Can you work these out from the model? Positions are in its coordinate system, mm. Give positions to 0.01 mm unless a question says otherwise; leave off trailing zeros. Loops run counter-clockwise (first coordinate to the right, second up) from the corner with the lowest first, then second, coordinate; pieces in that order, holes last. Notation, with made-up numbers: M -32.5,34.25 L -13.5,34.25 A22 cw -13.5,68.25 Z; hole C -8.5,10 d1. An arc over 180 degrees is marked long. Answer as a JSON object with one key per item and string values.
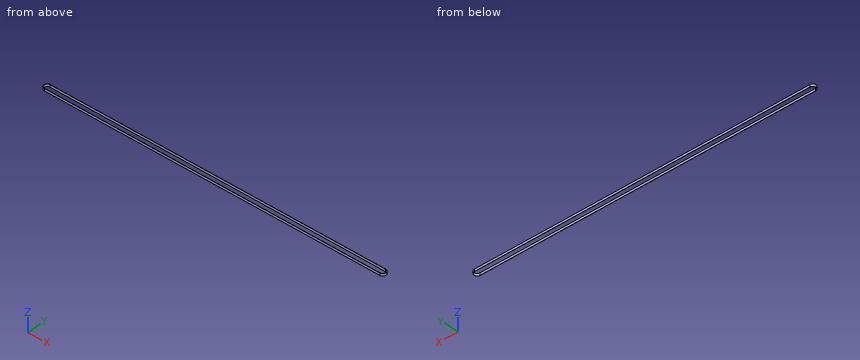
```python
from build123d import *

# Parameters (mm, degrees)
EXTRUDE_1_DEPTH = 7.5


with BuildPart() as part:
    # 草图2 → 拉伸-薄壁1 (new, symmetric)
    with BuildSketch(Plane.XY):
        with BuildLine():
            Line((2155, -20.415), (0, -20.415))
            ThreePointArc((0, -20.415), (-20.415, 0), (0, 20.415))
            Line((0, 20.415), (2155, 20.415))
            ThreePointArc((2155, 20.415), (2175.415, 0), (2155, -20.415))
        make_face()
        with BuildLine():
            Line((2155, -19.415), (0, -19.415))
            ThreePointArc((0, -19.415), (-19.415, 0), (0, 19.415))
            Line((0, 19.415), (2155, 19.415))
            ThreePointArc((2155, 19.415), (2174.415, 0), (2155, -19.415))
        make_face(mode=Mode.SUBTRACT)
    extrude(amount=EXTRUDE_1_DEPTH, both=True)


solid = part.part
```
1) Please list where these lines run through material, in increasing order: line 1 along Y through (x, z) = (229.5, -5.25) (3 decimals); line 2 along X through (y, z) = (-1.5, -5.5); line 3 along X through (y, z) = (2, 3.25). Write a range as from..to.
Answer list:
{"line 1": "-20.415..-19.415, 19.415..20.415", "line 2": "-20.36..-19.36, 2174.36..2175.36", "line 3": "-20.32..-19.31, 2174.31..2175.32"}
2) Will these pins go through, and if not, where does the flat tip stop? pin 1 Ø1 at (y, z) = (-8, 4) entering from +X; pin 2 Ø1 at (y, z) = (9, 0.5) entering from +X; pin 3 Ø5 at (y, z) = (-13, -1.5) entering from -X.
Answer list:
{"pin 1": "x = 2173.99", "pin 2": "x = 2173.56", "pin 3": "x = -17.51"}
3) Suppose I cut it at A-A, the plane z = -0.25. Write out the boundary of the cut face in (x, y) (3 decimals), and give its area (3 significant figures).
Answer list:
{"outline": "M 0,-20.415 L 2155,-20.415 A20.415 ccw 2155,20.415 L 0,20.415 A20.415 ccw Z; hole M 0,-19.415 L 2155,-19.415 A19.415 ccw 2155,19.415 L 0,19.415 A19.415 ccw Z", "area": "4,440 mm^2"}
4) Suppose I cut it at B-B, the plane y = -11. Write out the boundary of the cut face in (x, z).
Answer list:
{"outline": "M -17.2,-7.5 L -16,-7.5 L -16,7.5 L -17.2,7.5 Z; M 2171,-7.5 L 2172.2,-7.5 L 2172.2,7.5 L 2171,7.5 Z"}
5) Suppose I cut it at C-C, the plane x = 1839. Write out the boundary of the cut face in (y, z) (3 decimals).
Answer list:
{"outline": "M -20.415,-7.5 L -19.415,-7.5 L -19.415,7.5 L -20.415,7.5 Z; M 19.415,-7.5 L 20.415,-7.5 L 20.415,7.5 L 19.415,7.5 Z"}
